Read the model definition and answer for the solid it produces. Units are mm, in the model's axes. A direction names the side the tool comes from. Round coordinates to 2 decimals unless told otherwise and drop trailing zeros. Loops run counter-clockwise (first coordinate to the right, second up) from the corner with the lowest first, then second, coordinate; pieces in that order, holes last. Notation, with made-up numbers: M 58.25,-29.75 L 110.25,-29.75 A37 cw 110.25,6.25 Z; hole C 63.25,-10.75 d3. An arc over 180 degrees is marked long. Answer as CSV lines item,"result".
```python
from build123d import *

# Parameters (mm, degrees)
CLAMP_BODY_DEPTH             = 14
CLAMP_BORE_SKETCH_R          = 14
CLAMP_BORE_DEPTH             = 96
CLAMP_LUGS_DEPTH             = 28
SPLIT_SLOT_2MM_DEPTH         = 52
BODY_FILLET_R1_6_A_R         = 1.6
BODY_FILLET_R1_6_B_R         = 1.6
CLAMP_SCREW_HOLES_SKETCH_R   = 2
CLAMP_SCREW_HOLES_3X_DEPTH   = 52
SUPPORT_RIB_1_REACH          = 61.228
SUPPORT_RIB_1_SKETCH_WALL_W  = 145.754223634
SUPPORT_RIB_1_SKETCH_WALL_H  = 6
SUPPORT_RIB_2_REACH          = 61.228
SUPPORT_RIB_2_SKETCH_WALL_W  = 145.754223634
SUPPORT_RIB_2_SKETCH_WALL_H  = 6
BASE_MOUNTING_HOLES_SKETCH_R = 2
BASE_MOUNTING_HOLES_4X_DEPTH = 52
LUG_FILLET_R0_8_A_R          = 0.8
LUG_FILLET_R0_8_B_R          = 0.8
LUG_FILLET_R0_8_C_R          = 0.8
LUG_FILLET_R0_8_D_R          = 0.8


with BuildPart() as part:
    # Clamp Body Profile → Clamp Body (new, symmetric)
    with BuildSketch(Plane.XY):
        with BuildLine():
            Line((20, 24), (20, 0))
            Line((20, 0), (28, 0))
            Line((28, 0), (28, -6))
            Line((28, -6), (15.6, -6))
            Line((15.6, -6), (15.6, -4.4))
            Line((15.6, -4.4), (14, -4.4))
            Line((14, -4.4), (14, 9.717143143))
            ThreePointArc((14, 9.717143143), (0, 4), (-14, 9.717143143))
            Line((-14, 9.717143143), (-14, -4.4))
            Line((-14, -4.4), (-15.6, -4.4))
            Line((-15.6, -4.4), (-15.6, -6))
            Line((-15.6, -6), (-28, -6))
            Line((-28, -6), (-28, 0))
            Line((-28, 0), (-20, 0))
            Line((-20, 0), (-20, 24))
            ThreePointArc((-20, 24), (0, 44), (20, 24))
        make_face()
    extrude(amount=CLAMP_BODY_DEPTH, both=True)

    # Clamp Bore Sketch → Clamp Bore (cut)
    with BuildSketch(Plane.XY.offset(14)):
        with Locations((0, 24)):
            Circle(CLAMP_BORE_SKETCH_R)
    extrude(amount=-CLAMP_BORE_DEPTH, mode=Mode.SUBTRACT)

    # Clamp Lugs Sketch → Clamp Lugs (add)
    with BuildSketch(Plane.XY.offset(14)):
        Polygon((0, 38), (7, 38), (7, 42.734993995), (7, 50.278784028), (-7, 50.278784028), (-7, 38), align=None)
    extrude(amount=-CLAMP_LUGS_DEPTH)

    # Split Slot Sketch → Split Slot 2mm (cut)
    with BuildSketch(Plane.XY.offset(14)):
        Polygon((-1, 37.964240044), (-1, 37.406271495), (1, 37.406271495), (1, 38), (1, 50.278784028), (-1, 50.278784028), align=None)
    extrude(amount=-SPLIT_SLOT_2MM_DEPTH, mode=Mode.SUBTRACT)

    # Body Fillet R1.6 A
    body_fillet_r1_6_a_edges = [part.edges().sort_by_distance(p)[0] for p in [
        (20, 0, 0),
    ]]
    fillet(body_fillet_r1_6_a_edges, radius=BODY_FILLET_R1_6_A_R)

    # Body Fillet R1.6 B
    body_fillet_r1_6_b_edges = [part.edges().sort_by_distance(p)[0] for p in [
        (-20, 0, 0),
    ]]
    fillet(body_fillet_r1_6_b_edges, radius=BODY_FILLET_R1_6_B_R)

    # Clamp Screw Holes Sketch → Clamp Screw Holes 3x (cut)
    with BuildSketch(Plane(origin=(7, 0, 0), x_dir=(0, 0, -1), z_dir=(1, 0, 0))):
        with Locations((8.5, 46.678784028)):
            Circle(CLAMP_SCREW_HOLES_SKETCH_R)
        with Locations((-8.5, 46.678784028)):
            Circle(CLAMP_SCREW_HOLES_SKETCH_R)
        with Locations((0, 46.678784028)):
            Circle(CLAMP_SCREW_HOLES_SKETCH_R)
    extrude(amount=-CLAMP_SCREW_HOLES_3X_DEPTH, mode=Mode.SUBTRACT)

    # Support Rib 1 Sketch wall → Support Rib 1 (add, up to next)
    with BuildSketch(Plane(origin=(24, 12, 0), x_dir=(-0.316227766017, 0.948683298051, 0), z_dir=(-0.948683298051, -0.316227766017, 0)), mode=Mode.PRIVATE) as support_rib_1_sk1:
        Rectangle(SUPPORT_RIB_1_SKETCH_WALL_W, SUPPORT_RIB_1_SKETCH_WALL_H)
    support_rib_1_tool1 = extrude(support_rib_1_sk1.sketch, amount=SUPPORT_RIB_1_REACH, mode=Mode.PRIVATE) - part.part
    add(support_rib_1_tool1.solids().sort_by_distance((24, 12, 0))[0])

    # Support Rib 2 Sketch wall → Support Rib 2 (add, up to next)
    with BuildSketch(Plane(origin=(-24, 12, 0), x_dir=(-0.316227766017, -0.948683298051, 0), z_dir=(0.948683298051, -0.316227766017, 0)), mode=Mode.PRIVATE) as support_rib_2_sk1:
        Rectangle(SUPPORT_RIB_2_SKETCH_WALL_W, SUPPORT_RIB_2_SKETCH_WALL_H)
    support_rib_2_tool1 = extrude(support_rib_2_sk1.sketch, amount=SUPPORT_RIB_2_REACH, mode=Mode.PRIVATE) - part.part
    add(support_rib_2_tool1.solids().sort_by_distance((-24, 12, 0))[0])

    # Base Mounting Holes Sketch → Base Mounting Holes 4x (cut)
    with BuildSketch(Plane(origin=(0, 0, 0), x_dir=(1, 0, 0), z_dir=(0, 1, 0))):
        with Locations(Location((24.8, 8.5, 0), (0, 0, 180))):
            Circle(BASE_MOUNTING_HOLES_SKETCH_R)
        with Locations(Location((24.8, -8.5, 0), (0, 0, 180))):
            Circle(BASE_MOUNTING_HOLES_SKETCH_R)
        with Locations(Location((-24.8, 8.5, 0), (0, 0, 180))):
            Circle(BASE_MOUNTING_HOLES_SKETCH_R)
        with Locations(Location((-24.8, -8.5, 0), (0, 0, 180))):
            Circle(BASE_MOUNTING_HOLES_SKETCH_R)
    extrude(amount=-BASE_MOUNTING_HOLES_4X_DEPTH, mode=Mode.SUBTRACT)

    # Lug Fillet R0.8 A
    lug_fillet_r0_8_a_edges = [part.edges().sort_by_distance(p)[0] for p in [
        (4, 50.278784028, 14),
    ]]
    fillet(lug_fillet_r0_8_a_edges, radius=LUG_FILLET_R0_8_A_R)

    # Lug Fillet R0.8 B
    lug_fillet_r0_8_b_edges = [part.edges().sort_by_distance(p)[0] for p in [
        (-4, 50.278784028, 14),
    ]]
    fillet(lug_fillet_r0_8_b_edges, radius=LUG_FILLET_R0_8_B_R)

    # Lug Fillet R0.8 C
    lug_fillet_r0_8_c_edges = [part.edges().sort_by_distance(p)[0] for p in [
        (-4, 50.278784028, -14),
    ]]
    fillet(lug_fillet_r0_8_c_edges, radius=LUG_FILLET_R0_8_C_R)

    # Lug Fillet R0.8 D
    lug_fillet_r0_8_d_edges = [part.edges().sort_by_distance(p)[0] for p in [
        (4, 50.278784028, -14),
    ]]
    fillet(lug_fillet_r0_8_d_edges, radius=LUG_FILLET_R0_8_D_R)


solid = part.part
```
1) Find section A-A, the plane x = -24.8. Give the vertices of the cut face in (y, z), then the cut area to 3 significant figures.
Evaluation:
outline,"M -6,-14 L 0,-14 L 0,-10.5 L -6,-10.5 Z; M -6,-6.5 L 0,-6.5 L 0,-3 L 9.6,-3 L 9.6,3 L 0,3 L 0,6.5 L -6,6.5 Z; M -6,10.5 L 0,10.5 L 0,14 L -6,14 Z"
area,"178 mm^2"
2) Find section C-C, the plane z = 0. Count the separate pieces of the cut face and the enclosed holes in it, then the cut area to 3 significant figures.
Evaluation:
separate pieces,"3"
enclosed holes,"0"
area,"1,190 mm^2"
3) Find section B-B, the plane z = -5.25. Give the vertices of the cut face in (x, y) (3 decimals), then the cut area to 3 significant figures.
Evaluation:
outline,"M -28,-6 L -15.6,-6 L -15.6,-4.4 L -14,-4.4 L -14,9.717 A20 ccw 14,9.717 L 14,-4.4 L 15.6,-4.4 L 15.6,-6 L 28,-6 L 28,0 L 21.6,0 A1.6 cw 20,1.6 L 20,24 A20 ccw 7,42.735 L 7,50.279 L 1,50.279 L 1,37.964 A14 cw long -1,37.964 L -1,50.279 L -7,50.279 L -7,42.735 A20 ccw -20,24 L -20,1.6 A1.6 cw -21.6,0 L -28,0 Z"
area,"1,040 mm^2"
4) Find section D-D, the plane y = 36. Give the vertices of the cut face in (x, z).
Evaluation:
outline,"M -16,-14 L -7.21,-14 L -7.21,14 L -16,14 Z; M 7.21,-14 L 16,-14 L 16,14 L 7.21,14 Z"
5) Determine the mould class of faces 5 (the cylindrical face through (-3.958, 45.462, 10.087)), 6 (the flat face through (15.6, -5, 0)), 7 (the flat face through (7, 44, 0)) for opening direction X: released by +X, released by -X, zero draft, split by the parting line, or undercut.
Evaluation:
face 5,"zero draft"
face 6,"undercut"
face 7,"released by +X"
6) Straight lines are drawn through the part: line 1 (X direction, y = 43, z = 9.25); line 2 (Y direction, x = -2, z = -7.75); line 3 (X direction, y = 8.5, z = -7.5). For each, find the intervals that lie inside material, in ascending order.
Evaluation:
line 1,"x = -7 to -1, 1 to 7"
line 2,"y = 4.1 to 10.14, 37.86 to 44.82, 48.53 to 50.28"
line 3,"x = -20 to -14, -12.64 to 12.64, 14 to 20"
7) A tool of negligible diameter and unlimited length cuts with its end or side. For faces 1 (the flat face through (-22, 9, 3)), 2 (the flat face through (-15.6, -5, 0)), 3 (the flat face through (22, 8, -3)), 4 (the flat face through (-20, 13, -8)), from which of +Z, -Z, +X, -X, +Y, -Y can it reach the whole face along a straight path? Write none if from no direction.
Evaluation:
face 1,"+Z, -X, +Y"
face 2,"+Z, -Z, -Y"
face 3,"-Z, +X, +Y"
face 4,"-Z, -X, +Y"
8) Each of these flat-tipped pins is pushed along its axis until it touches: P1, Ø3, axis at x = 5.5, y = 33.5, coming from the -Z side; P2, Ø6.5, axis at y = 46.68, z = 8.5, coming from the +X side; P3, Ø4.5, axis at x = -24.8, z = -8.5, coming from the +Y side; P4, Ø4, axis at x = -22.5, y = 15.5, coming from the -Z side. Where does it stop, or does it pass through?
Evaluation:
P1,"passes through"
P2,"stops at x = 7"
P3,"stops at y = 0"
P4,"stops at z = -3"
